```python
from build123d import *

# Parameters (mm, degrees)
SKETCH1_W           = 7.9
SKETCH1_H           = 7.8
BOSS_EXTRUDE1_DEPTH = 8
FILLET1_R           = 1
BOSS_EXTRUDE2_REACH = 22.756
SKETCH4_R           = 3.3
SKETCH6_R           = 3.925
BOSS_EXTRUDE3_DEPTH = 6.75
SKETCH9_R           = 3.1
CUT_EXTRUDE1_DEPTH  = 5


with BuildPart() as part:
    # Sketch1 → Boss-Extrude1 (new body)
    with BuildSketch(Plane(origin=(0, 0, 0), x_dir=(1, 0, 0), z_dir=(0, 1, 0))):
        Rectangle(SKETCH1_W, SKETCH1_H)
    extrude(amount=BOSS_EXTRUDE1_DEPTH)

    # Fillet1
    fillet1_edges = [part.edges().sort_by_distance(p)[0] for p in [
        (-3.95, 8, 0),
        (3.95, 8, 0),
        (-3.95, 0, 0),
        (3.95, 0, 0),
    ]]
    fillet(fillet1_edges, radius=FILLET1_R)

    # Sketch3 → Cut-Revolve4 (revolve, cut)
    with BuildSketch(Plane(origin=(-2, 2, 0), x_dir=(0, 0, -1), z_dir=(0.7071067811865462, -0.7071067811865488, 0))):
        Polygon((3, 8.228427125), (4, 8.228427125), (3.9, 6.828427125), align=None)
    cut_revolve4 = revolve(axis=Axis((0, 4, 3.9), (0, 0, -1)), mode=Mode.SUBTRACT)

    # Mirror2: Cut-Revolve4 across plane
    add(cut_revolve4.mirror(Plane.XY), mode=Mode.SUBTRACT)

    # Sketch4 → Boss-Extrude2 (add, up to next)
    with BuildSketch(Plane(origin=(0, 20, 0), x_dir=(1, 0, 0), z_dir=(0, 1, 0)), mode=Mode.PRIVATE) as boss_extrude2_sk1:
        with Locations(Location((0, 0, 0), (0, 0, 270))):
            Circle(SKETCH4_R)
    boss_extrude2_tool1 = extrude(boss_extrude2_sk1.sketch, amount=-BOSS_EXTRUDE2_REACH, mode=Mode.PRIVATE) - part.part
    add(boss_extrude2_tool1.solids().sort_by_distance((0, 20, 0))[0])

    # Sketch5 → Revolve1 (revolve)
    with BuildSketch(Plane(origin=(0, 0, 0), x_dir=(0, 0, -1), z_dir=(1, 0, 0)), mode=Mode.PRIVATE) as revolve1_sk:
        Polygon((-5.1, 11), (-5.1, 9.8), (-3.3, 9.8), (-3.3, 15), (-3.95, 15), (-3.95, 12.25), (-3.4, 12.25), (-3.4, 11), align=None)
    revolve(revolve1_sk.sketch.rotate(Axis((0, -3.247015834, 0), (0, 1, 0)), 180), axis=Axis((0, -3.247015834, 0), (0, 1, 0)))

    # Sketch6 → Boss-Extrude3 (add)
    with BuildSketch(Plane(origin=(0, 0, -3.9), x_dir=(-1, 0, 0), z_dir=(0, 0, -1))):
        with Locations(Location((0, 4, 0), (0, 0, 180))):
            Circle(SKETCH6_R)
    extrude(amount=BOSS_EXTRUDE3_DEPTH)

    # Sketch8 → Revolve2 (revolve)
    with BuildSketch(Plane(origin=(0, 0, 0), x_dir=(0, 0, -1), z_dir=(1, 0, 0)), mode=Mode.PRIVATE) as revolve2_sk:
        Polygon((5.3, 4), (5.3, 8.95), (12.4, 8.95), (12.4, 8.575), (13.9, 8.575), (13.9, 7.6875), (13.4, 7.6875), (12.887601636, 6.8), (10.65, 6.8), (10.65, 4.470320629), (12.385380774, 4.470320629), (13.2, 4), align=None)
    revolve(revolve2_sk.sketch.rotate(Axis((0, 4, 5.444048586), (0, 0, -1)), 90), axis=Axis((0, 4, 5.444048586), (0, 0, -1)))

    # Sketch9 → Cut-Extrude1 (cut)
    with BuildSketch(Plane.XY.offset(3.9)):
        with Locations((0, 4)):
            Circle(SKETCH9_R)
    extrude(amount=-CUT_EXTRUDE1_DEPTH, mode=Mode.SUBTRACT)


solid = part.part
```
Here's how the part is built. I have some questions about the finished solid (model axes, mm). A direction names the side the tool comes from. Give positions to 0.01 mm unless a question says otherwise; leave off trailing zeros. Loops run counter-clockwise (first coordinate to the right, second up) from the corner with the lowest first, then second, coordinate; pieces in that order, holes last. Notation, with made-up numbers: (15, 1.5) -> (38, 1.5) arc R12 cw to (38, 6.5) -> close; hole circle Ø1 at (80, -5.5). An arc over 180 degrees is marked (long way). Use one line per item in the form item = value. Start each with the question number.
1) Imagine slicing it at C-C (z = -7.5). Please give me the cut outline in (x, y), then the cut area to 3 significant figures.
2) Thinking about a two-plate mould opening in Y: for faces 1 (the face through (-2.79, 0.67, -3.68)), 2 (the face through (-0.992, 8.466, -13.16)), 3 (the face through (-0.48, 0.344, -13.646)), 4 (the face through (0, 0, -13.9)), which applies, +Y half, -Y half, draft (parallel to the pull), parting line (faces both ways), or undercut?
3) Please list where these lines run through material, in increasing order: line 1 along Y through (x, z) = (0, -13.55) (1 decimal); line 2 along Z through (x, y) = (0.25, 5.5); line 3 along Y through (x, z) = (3.75, -2.5).
4) Imagine slicing it at A-A (z = 0). Please give me the cut outline in (x, y).
5) Which directions (+Z, -Z, +X, -X, +Y, -Y) give clear straight access to the entire face, cutting with the end or side of a thin tool? Please do faces 5 (the face through (0, 4, -1.1)), 6 (the face through (2.79, 7.33, 3.68)), 7 (the face through (3.95, 4, 0)).
6) For P1, Ø4, axis at x = 1, y = 6, coming from the +Z side; P2, Ø6, axis at y = 11, z = -2, coming from the +X side; P3, Ø5, axis at x = 3, y = 17.5, coming from the +Z side; P4, Ø1, axis at x = 1.5, z = 0.5, coming from the -Y side, each with a flat end and sliding along its axis, tell me the tip position at first contact or that it passes through.
7) Imagine slicing it at B-B (y = 11.75). Please give me the cut outline in (x, z).
Check values:
q1.outline = circle Ø9.9 at (0, 4)
q1.area = 77.0 mm^2
q2.face_1 = -Y half
q2.face_2 = parting line
q2.face_3 = undercut
q2.face_4 = draft
q3.line_1 = -0.6 to 0.3, 7.7 to 8.6
q3.line_2 = -10.65 to -1.1
q3.line_3 = 0.4 to 7.6, 9.8 to 11
q4.outline = (-5.1, 9.8) -> (-3.3, 9.8) -> (-3.3, 7.94) arc R1 ccw to (-3.95, 7) -> (-3.95, 1) arc R1 ccw to (-2.95, 0) -> (2.95, 0) arc R1 ccw to (3.95, 1) -> (3.95, 7) arc R1 ccw to (3.3, 7.94) -> (3.3, 9.8) -> (5.1, 9.8) -> (5.1, 11) -> (3.4, 11) -> (3.4, 12.25) -> (3.95, 12.25) -> (3.95, 15) -> (3.3, 15) -> (3.3, 20) -> (-3.3, 20) -> (-3.3, 15) -> (-3.95, 15) -> (-3.95, 12.25) -> (-3.4, 12.25) -> (-3.4, 11) -> (-5.1, 11) -> close; hole circle Ø6.2 at (0, 4)
q5.face_5 = +Z
q5.face_6 = +Z, +X
q5.face_7 = +Z, +X, -Y
q6.P1 = 3.9
q6.P2 = 5.1
q6.P3 = 3.26
q6.P4 = 0
q7.outline = circle Ø6.8 at (0, 0)
